Could you check a few things on this model? Use its own coordinates, in mm. A direction names the side the tool comes from. Round coordinates to 2 decimals unless told otherwise and drop trailing zeros. Order: outer loops, then holes, each group sorted by start corner. A loop starts at its lowest first (then second) coordinate and runs counter-clockwise, first axis right, second up. Notation, with made-up numbers: M -13,24 L 22,24 A21 ccw 22,62 Z; hole C 20.25,50.25 d7. An arc over 180 degrees is marked long. Write each question's results on one line, items separated by ' | '. Start each with the question number.
1. Suppose I cut it at B-B on x = -60. Write out the boundary of the cut face in (y, z), and give its area (3 significant figures).
2. Please list where these lines run through material, in increasing order: L1, parallel to X at y = 5, z = 452; L2, parallel to Y at x = -69, z = 453.5.
3. For faces 1 (the flat face through (-79, 3, 0)), 2 (the flat face through (-65, 24.825, 317)), which set-ups out of +Z, -Z, +X, -X, +Y, -Y let a thin tool reach every point of the face, with its end or its side?
4. Suppose I cut it at A-A on y = 13.5. Write out the boundary of the cut face in (x, z).
5. Suppose I cut it at C-C on z = 549.5. Write out the boundary of the cut face in (x, y).
6. We'd pull the mould along Y, two halves only. Please class faces 3 (the flat face through (-79, 3, 644)), 4 (the flat face through (-65, 26.825, 317)), 5 (the flat face through (-65, -24.284, 317)), 6 (the flat face through (-50.989, 1, 317)): released by +Y, released by -Y, zero draft, split by the parting line, or undercut.
from build123d import *

# Parameters (mm, degrees)
SKETCH1_W           = 31.515629069
SKETCH1_H           = 51.109180057
SKETCH1_W_2         = 27.515629069
SKETCH1_H_2         = 47.109180057
BOSS_EXTRUDE1_DEPTH = 644


with BuildPart() as part:
    # Sketch1 → Boss-Extrude1 (new body)
    with BuildSketch(Plane.XY):
        with Locations((-64.747167395, 1.270489558)):
            Rectangle(SKETCH1_W, SKETCH1_H)
        with Locations((-64.747167395, 1.270489558)):
            Rectangle(SKETCH1_W_2, SKETCH1_H_2, mode=Mode.SUBTRACT)
    extrude(amount=BOSS_EXTRUDE1_DEPTH)


solid = part.part
Filled sheet:
1) outline: M -24.28,0 L -22.28,0 L -22.28,644 L -24.28,644 Z; M 24.83,0 L 26.83,0 L 26.83,644 L 24.83,644 Z | area: 2,580 mm^2
2) L1: x = -80.5 to -78.5, -50.99 to -48.99 | L2: y = -24.28 to -22.28, 24.83 to 26.83
3) face 1: -Z, +X, -X, +Y, -Y | face 2: +Z, -Z
4) outline: M -80.5,0 L -78.5,0 L -78.5,644 L -80.5,644 Z; M -50.99,0 L -48.99,0 L -48.99,644 L -50.99,644 Z
5) outline: M -80.5,-24.28 L -48.99,-24.28 L -48.99,26.83 L -80.5,26.83 Z; hole M -78.5,-22.28 L -50.99,-22.28 L -50.99,24.83 L -78.5,24.83 Z
6) face 3: zero draft | face 4: released by +Y | face 5: released by -Y | face 6: undercut
